Could you check a few things on this model? Use its own coordinates, in mm. A direction names the side the tool comes from. Give positions to 0.01 mm unless a question says otherwise; leave off trailing zeros. Order: outer loops, then holes, each group sorted by start corner. A loop starts at its lowest first (then second) coordinate and runs counter-clockwise, first axis right, second up. Notation, with made-up numbers: M 89,68 L 110,68 A19 ccw 110,77 Z; hole C 67.5,79.5 d2. An arc over 180 degrees is marked long. Use a Markdown table: item, result. Add a question column.
Item 1: For faces 1 (the face through (-89.313, 9.86, 79.142)), 2 (the face through (0.97, 9.86, -96.995)), which set-ups out of +Z, -Z, +X, -X, +Y, -Y let a thin tool reach every point of the face, with its end or its side?
Item 2: Suppose I cut it at D-D on x = 72.5. Write out the boundary of the cut face in (y, z).
Item 3: Suppose I cut it at A-A on z = -43.5. Write out the boundary of the cut face in (x, y), plus the area to 3 significant figures.
Item 4: If I drill on L1, parallel to X at y = 17.5, z = 7.5; L2, parallel to Z at x = -2, y = 7.5; L3, parallel to Z at x = -64, y = 12.75, over which ranges is the centre line in solid material (lowest first)? Write a range as from..to.
Item 5: If we mould it in two halves opening along Z, with no side actions, what happens to faces 3 (the face through (-66.072, 10.14, -69.933)), 4 (the face through (-1.368, 9.86, 119.992)), 5 (the face through (-90, 10, -1)), 6 (the face through (-89.274, 9.86, -79.24))? For each: released by +Z, released by -Z, zero draft, split by the parting line, or undercut.
Item 6: Suppose I cut it at C-C on x = 16. Write out the boundary of the cut face in (y, z), plus the area to 3 significant figures.
Item 7: Suppose I cut it at B-B on y = 2.5. Write out the boundary of the cut face in (x, z), plus the area to 3 significant figures.
Item 8: I'm going to push flat-ended pins straight in: pin 1 Ø4 at (x, y) = (-65, 14.5) entering from -Z; pin 2 Ø1.5 at (x, y) = (66, 9) entering from -Z; pin 3 Ø10 at (x, y) = (62.5, 6.5) entering from -Z. Where does each tip first touch, or does it pass through?
from build123d import *

# Parameters (mm, degrees)
EXTRUDE_1_DEPTH = 20
FILLET_1_R      = 10


with BuildPart() as part:
    # 草图1 → 凸台-拉伸1 (new body)
    with BuildSketch(Plane(origin=(0, 0, 0), x_dir=(1, 0, 0), z_dir=(0, 1, 0))):
        with BuildLine():
            Line((90, -75.498344353), (90, 75.498344353))
            ThreePointArc((90, 75.498344353), (89.293203773, 79.191089082), (87.272727273, 82.361830203))
            ThreePointArc((87.272727273, 82.361830203), (0, 120), (-87.272727273, 82.361830203))
            ThreePointArc((-87.272727273, 82.361830203), (-89.293203773, 79.191089082), (-90, 75.498344353))
            Line((-90, 75.498344353), (-90, -75.498344353))
            ThreePointArc((-90, -75.498344353), (-89.293203773, -79.191089082), (-87.272727273, -82.361830203))
            ThreePointArc((-87.272727273, -82.361830203), (0, -120), (87.272727273, -82.361830203))
            ThreePointArc((87.272727273, -82.361830203), (89.293203773, -79.191089082), (90, -75.498344353))
        make_face()
        with BuildLine():
            Line((67, -70.142711667), (67, 70.142711667))
            ThreePointArc((67, 70.142711667), (0, 97), (-67, 70.142711667))
            Line((-67, 70.142711667), (-67, -70.142711667))
            ThreePointArc((-67, -70.142711667), (0, -97), (67, -70.142711667))
        make_face(mode=Mode.SUBTRACT)
    extrude(amount=EXTRUDE_1_DEPTH)

    # 圆角1
    fillet_1_edges = [part.edges().sort_by_distance(p)[0] for p in [
        (-67, 10, 70.142711667),
        (67, 10, 70.142711667),
        (67, 10, -70.142711667),
        (-67, 10, -70.142711667),
    ]]
    fillet(fillet_1_edges, radius=FILLET_1_R)


solid = part.part
Findings below:
| question | item | result |
|---|---|---|
| 1 | face 1 | +Z, -X, +Y, -Y |
| 1 | face 2 | +Y, -Y |
| 2 | outline | M 0,-95.62 L 20,-95.62 L 20,95.62 L 0,95.62 Z |
| 3 | outline | M -90,0 L -67,0 L -67,20 L -90,20 Z; M 67,0 L 90,0 L 90,20 L 67,20 Z |
| 3 | area | 920 mm^2 |
| 4 | L1 | x = -90..-67, 67..90 |
| 4 | L2 | z = -119.98..-96.98, 96.98..119.98 |
| 4 | L3 | z = -101.51..-72.87, 72.87..101.51 |
| 5 | face 3 | undercut |
| 5 | face 4 | released by +Z |
| 5 | face 5 | zero draft |
| 5 | face 6 | released by -Z |
| 6 | outline | M 0,-118.93 L 20,-118.93 L 20,-95.67 L 0,-95.67 Z; M 0,95.67 L 20,95.67 L 20,118.93 L 0,118.93 Z |
| 6 | area | 930 mm^2 |
| 7 | outline | M -90,-75.5 A10 ccw -87.27,-82.36 A120 ccw 87.27,-82.36 A10 ccw 90,-75.5 L 90,75.5 A10 ccw 87.27,82.36 A120 ccw -87.27,82.36 A10 ccw -90,75.5 Z; hole M -67,-65.73 A10 ccw -63.55,-73.28 A97 ccw 63.55,-73.28 A10 ccw 67,-65.73 L 67,65.73 A10 ccw 63.55,73.28 A97 ccw -63.55,73.28 A10 ccw -67,65.73 Z |
| 7 | area | 15,000 mm^2 |
| 8 | pin 1 | stops at z = -102.13 |
| 8 | pin 2 | stops at z = -100.71 |
| 8 | pin 3 | stops at z = -105.33 |
